Here's how the part is built. I have some questions about the finished solid (model axes, mm). Face numbers are marked on the shaded views. A direction names the side the tool comes from. Coordinates: 2 decimals unless noted, no trailing zeros. Write each loop counter-clockwise with the first axis right and the second up, starting at its lowest first coordinate (ties: lowest second). Pieces come first, ordered by that corner, then holes.
Item 1: If we section it at B-B (z = 0): Please give me the cut outline in (x, y), then the cut area to 3 significant figures.
Item 2: I'm going to push flat-ended pins straight in: pin 1 Ø10 at (y, z) = (16.5, 9.5) entering from +X; pin 2 Ø1 at (x, y) = (-5, 12.5) entering from +Z; pin 3 Ø13 at (y, z) = (13.94, 0) entering from -X. Where does each tip first touch, or does it pass through?
Item 3: If we section it at C-C (x = 2.25): Please give me the cut outline in (y, z).
Item 4: We'd pull the mould along X, two halves only. Please class the marked faces 1, 2, 3 and 4: +X half, -X half, draft (parallel to the pull), parting line (faces both ways), or undercut.
Item 5: If I drill on line 1 (Y direction, x = -4.95, z = 0); line 2 (X direction, y = 9, z = -0.5); line 3 (Y direction, x = -11.25, z = -5.5), over which ranges is the centre line in solid material (lowest first)?
Item 6: For the marked faces 5 and 6, which set-ups out of +Z, -Z, +X, -X, +Y, -Y let a thin tool reach every point of the face, with its end or its side?
Item 7: If we section it at A-A (y = 7.5): Please give me the cut outline in (x, z).
Item 8: If we section it at D-D (z = 6.5): Please give me the cut outline in (x, y).
from build123d import *

# Parameters (mm, degrees)
BOSS_EXTRU_1_DEPTH = 4
SKETCH2_W          = 2
SKETCH2_H          = 21.522663516
BOSS_EXTRU_2_DEPTH = 18
FILLET1_R          = 6
SKETCH3_R          = 4
CUT_EXTRUDE1_DEPTH = 34.707714251


with BuildPart() as part:
    # Sketch1 → Boss.-Extru.1 (new body)
    with BuildSketch(Plane(origin=(0, 0, 0), x_dir=(1, 0, 0), z_dir=(0, 1, 0))):
        with BuildLine():
            Line((-8.5, -17.5), (8.5, -17.5))
            ThreePointArc((8.5, -17.5), (11.328427125, -16.328427125), (12.5, -13.5))
            Line((12.5, -13.5), (12.5, 13.5))
            ThreePointArc((12.5, 13.5), (11.328427125, 16.328427125), (8.5, 17.5))
            Line((8.5, 17.5), (-8.5, 17.5))
            ThreePointArc((-8.5, 17.5), (-11.328427125, 16.328427125), (-12.5, 13.5))
            Line((-12.5, 13.5), (-12.5, -13.5))
            ThreePointArc((-12.5, -13.5), (-11.328427125, -16.328427125), (-8.5, -17.5))
        make_face()
    extrude(amount=BOSS_EXTRU_1_DEPTH)

    # Sketch2 → Boss.-Extru.2 (add)
    with BuildSketch(Plane(origin=(0, 4, 0), x_dir=(1, 0, 0), z_dir=(0, 1, 0))):
        with Locations((-5.1, 0)):
            Rectangle(SKETCH2_W, SKETCH2_H)
        with Locations((5.1, 0)):
            Rectangle(SKETCH2_W, SKETCH2_H)
    extrude(amount=BOSS_EXTRU_2_DEPTH)

    # Fillet1
    fillet1_edges = [part.edges().sort_by_distance(p)[0] for p in [
        (5.1, 22, -10.761331758),
        (5.1, 22, 10.761331758),
        (-5.1, 22, -10.761331758),
        (-5.1, 22, 10.761331758),
    ]]
    fillet(fillet1_edges, radius=FILLET1_R)

    # Sketch3 → Cut-Extrude1 (cut, through all)
    with BuildSketch(Plane(origin=(6.1, 0, 0), x_dir=(0, 0, -1), z_dir=(1, 0, 0))):
        with Locations((0, 13.939258033)):
            Circle(SKETCH3_R)
    extrude(amount=-CUT_EXTRUDE1_DEPTH, mode=Mode.SUBTRACT)


solid = part.part
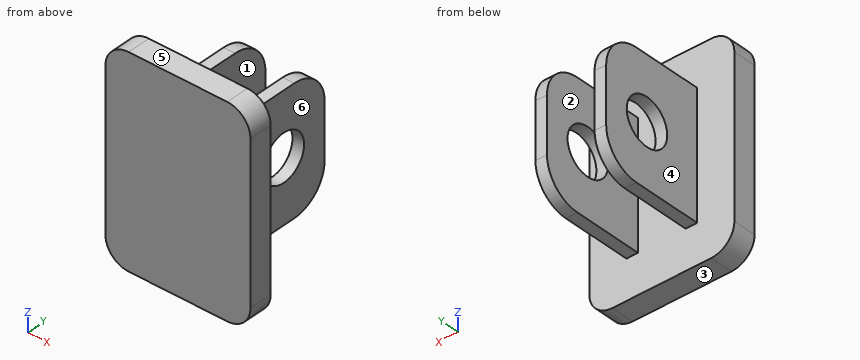
Answer list:
1. outline: (-12.5, 0) - (12.5, 0) - (12.5, 4) - (6.1, 4) - (6.1, 9.94) - (4.1, 9.94) - (4.1, 4) - (-4.1, 4) - (-4.1, 9.94) - (-6.1, 9.94) - (-6.1, 4) - (-12.5, 4) - close; (-6.1, 17.94) - (-4.1, 17.94) - (-4.1, 22) - (-6.1, 22) - close; (4.1, 17.94) - (6.1, 17.94) - (6.1, 22) - (4.1, 22) - close
1. area: 140 mm2
2. pin 1: stops at x = 6.1
2. pin 2: stops at z = 10.76
2. pin 3: stops at x = -6.1
3. outline: (0, -17.5) - (4, -17.5) - (4, 17.5) - (0, 17.5) - close
4. face 1: undercut
4. face 2: undercut
4. face 3: draft
4. face 4: -X half
5. line 1: y = 0 to 9.94, 17.94 to 22
5. line 2: x = -6.1 to -4.1, 4.1 to 6.1
5. line 3: y = 0 to 4
6. face 5: +Z, +X, -X, +Y, -Y
6. face 6: +Z, -Z, +X, +Y
7. outline: (-6.1, -10.76) - (-4.1, -10.76) - (-4.1, 10.76) - (-6.1, 10.76) - close; (4.1, -10.76) - (6.1, -10.76) - (6.1, 10.76) - (4.1, 10.76) - close
8. outline: (-12.5, 0) - (12.5, 0) - (12.5, 4) - (6.1, 4) - (6.1, 21.74) - (4.1, 21.74) - (4.1, 4) - (-4.1, 4) - (-4.1, 21.74) - (-6.1, 21.74) - (-6.1, 4) - (-12.5, 4) - close
